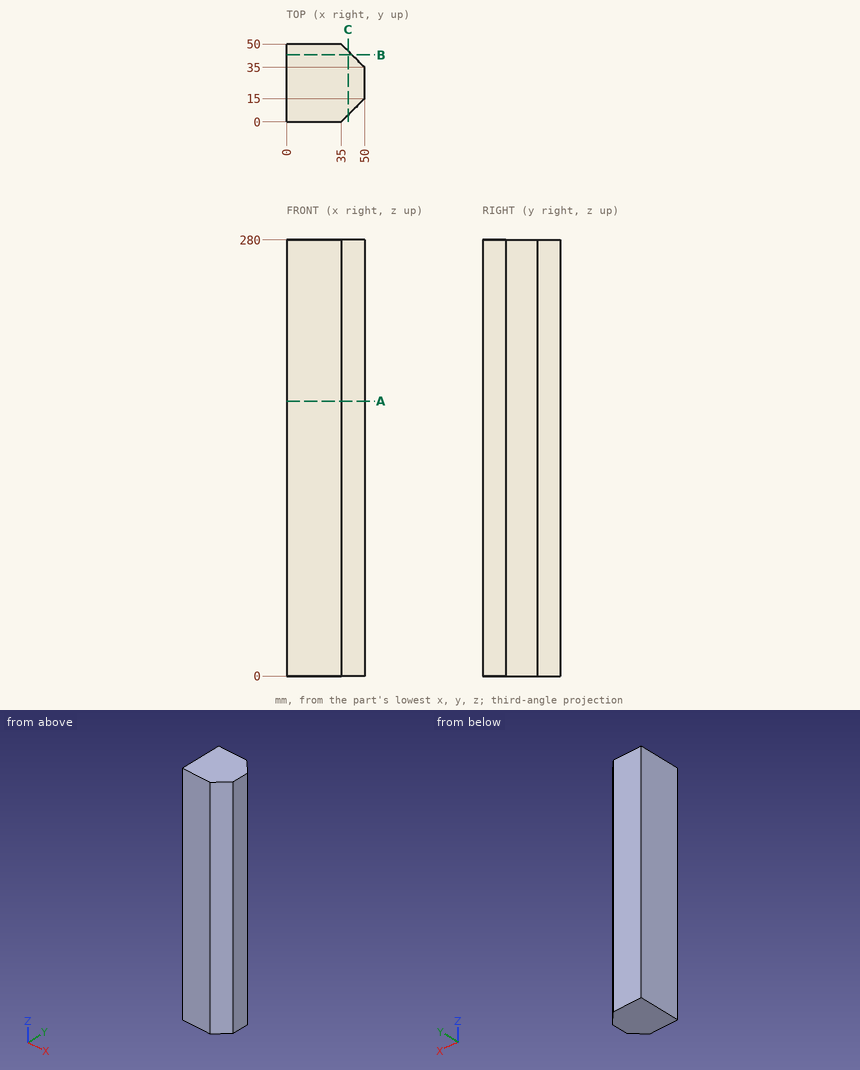
Could you check a few things on this drawing? It's one solid part, dimensions in mm from its lowest x, y, z. Give positions to 0.01 mm unless a question says otherwise; leave off trailing zeros. Loops run counter-clockwise (first coordinate to the right, second up) from the corner with the lowest first, then second, coordinate; pieces in that order, holes last. Notation, with made-up numbers: M -25.75,14.25 L 9.25,14.25 A16 cw 9.25,45.25 Z; hole C 26.5,-7.5 d11. An arc over 180 degrees is marked long. Answer as a JSON object with one key per item and string values.
Q1. Suppose I cut it at B-B, the plane y = 43. List the corners of the cut face in (x, z) for me, plus the area to 3 significant figures.
Values found:
{"outline": "M 0,0 L 42,0 L 42,280 L 0,280 Z", "area": "11,800 mm²"}
Q2. Suppose I cut it at C-C, the plane x = 39.5. List the corners of the cut face in (y, z) for me, plus the area to 3 significant figures.
Values found:
{"outline": "M 4.5,0 L 45.5,0 L 45.5,280 L 4.5,280 Z", "area": "11,500 mm²"}
Q3. If I drill on probe 1 along X at (y, z) = (14, 230.5); probe 2 along Y at (x, z) = (47.5, 112.5); probe 3 along Y at (x, z) = (41.5, 160), over which ranges is the centre line in solid material (lowest first)? Write a range as [from, to].
Values found:
{"probe 1": "x = [0, 49]", "probe 2": "y = [12.5, 37.5]", "probe 3": "y = [6.5, 43.5]"}
Q4. Suppose I cut it at A-A, the plane z = 176.5. List the corners of the cut face in (x, y) for me, plus the area to 4 significant figures.
Values found:
{"outline": "M 0,0 L 35,0 L 50,15 L 50,35 L 35,50 L 0,50 Z", "area": "2,275 mm²"}
Q5. For P1, Ø5, axis at x = 41.5, z = 98, coming from the +Y side; P2, Ø10, axis at x = 44.5, z = 102.5, coming from the +Y side; P3, Ø2, axis at x = 38.5, z = 241.5, coming from the -Y side, each with a flat end and sliding along its axis, tell me the tip position at first contact or that it passes through.
Values found:
{"P1": "stops at y = 46", "P2": "stops at y = 45.5", "P3": "stops at y = 2.5"}
